Geometry check sheet. Reference: the model listing, model coordinates, mm. A direction names the side the tool comes from. Give positions to 0.01 mm unless a question says otherwise; leave off trailing zeros. Loops run counter-clockwise (first coordinate to the right, second up) from the corner with the lowest first, then second, coordinate; pieces in that order, holes last. Notation, with made-up numbers: (-28, 65) - (26, 65) arc R26 cw to (26, 94) - close; hole circle Ø7 at (-18, -14.5). An arc over 180 degrees is marked (long way). Write item = value, one per line. Start each with the question number.
from build123d import *

# Parameters (mm, degrees)
SKETCH_1_W            = 90
SKETCH_1_H            = 25
EXTRUDE_1_DEPTH       = 12
SKETCH_2_W            = 40
SKETCH_2_H            = 25
EXTRUDE_2_DEPTH       = 35
HOLE_WIZARD_M20_1_D   = 17.5
HOLE_WIZARD_9_0_9_1_D = 9
CHAMFER_1_SIZE        = 5
CHAMFER_2_SIZE        = 3


with BuildPart() as part:
    # 草图1 → 凸台-拉伸1 (new body)
    with BuildSketch(Plane(origin=(0, 0, 0), x_dir=(0, 0, -1), z_dir=(1, 0, 0))):
        Rectangle(SKETCH_1_W, SKETCH_1_H)
    extrude(amount=EXTRUDE_1_DEPTH)

    # 草图2 → 凸台-拉伸2 (add)
    with BuildSketch(Plane(origin=(12, 0, 0), x_dir=(0, 0, -1), z_dir=(1, 0, 0))):
        Rectangle(SKETCH_2_W, SKETCH_2_H)
    extrude(amount=EXTRUDE_2_DEPTH)

    # M20 螺纹孔1 (through all)
    with Locations(Plane(origin=(0, -12.5, 0), x_dir=(-1, 0, 0), z_dir=(0, -1, 0))):
        with Locations((-30, 0)):
            Hole(HOLE_WIZARD_M20_1_D / 2)

    # Ø9.0 (9) 直径孔1 (through all)
    with Locations(Plane(origin=(12, 0, 0), x_dir=(0, 0, -1), z_dir=(1, 0, 0))):
        with Locations((-30, 0), (30, 0)):
            Hole(HOLE_WIZARD_9_0_9_1_D / 2)

    # 倒角1
    chamfer_1_edges = [part.edges().sort_by_distance(p)[0] for p in [
        (47, 0, -20),
        (47, 0, 20),
    ]]
    chamfer(chamfer_1_edges, length=CHAMFER_1_SIZE)

    # 倒角2
    chamfer_2_edges = [part.edges().sort_by_distance(p)[0] for p in [
        (6, -12.5, -45),
        (6, -12.5, 45),
        (6, 12.5, 45),
        (6, 12.5, -45),
    ]]
    chamfer(chamfer_2_edges, length=CHAMFER_2_SIZE)


solid = part.part
1) Material ranges on line 1 along Z through (x, y) = (30, -0.5); line 2 along Y through (x, z) = (8.75, -30); line 3 along Z through (x, y) = (6.5, -4), recorded low to high.
2) Cross-section at A-A on y = 0. Enter the section's corners in (x, z), and give its area (3 significant figures).
3) Cross-section at C-C on x = 28.5. Enter the section's corners in (y, z).
4) Release check for a two-part mould opening along Y. For faces 1 (the face through (5.916, 1.352, 34.292)), 2 (the face through (27, 0, -20)), 3 (the face through (18, 12.5, 1)) record: pulls with the +Y half, pulls with the -Y half, needs draft (parallel to the pull), parting line crosses it, or undercut.
5) Cross-section at B-B on z = 30. Enter the section's corners in (x, y), and give its area (3 significant figures).
6) Cross-section at D-D on x = 3. Enter the section's corners in (y, z), and give its area (3 significant figures).
7) Tool access check on faces 4 (the face through (27, 0, 20)), 5 (the face through (12, 0, -35)), 6 (the face through (6, 0, 45)). Record the directions out of +Z, -Z, +X, -X, +Y, -Y that give a thin tool (end or side, any length) a straight path to the whole face; none if there is none.
8) Gauge pin test, flat ends, axial feed: P1, Ø1, axis at x = 24, y = 2, coming from the +Z side; P2, Ø4, axis at x = 38, y = -2, coming from the -Z side; P3, Ø1.5, axis at y = 1, z = -22.5, coming from the +X side. Record the tip position at first contact, or that the pin passes through.
Checked values:
q1.line_1 = -20 to -8.75, 8.75 to 20
q1.line_2 = -12.5 to -4.5, 4.5 to 12.5
q1.line_3 = -45 to -32.06, -27.94 to 27.94, 32.06 to 45
q2.outline = (0, -45) - (12, -45) - (12, -34.5) - (0, -34.5) - close; (0, -25.5) - (12, -25.5) - (12, -20) - (42, -20) - (47, -15) - (47, 15) - (42, 20) - (12, 20) - (12, 25.5) - (0, 25.5) - close; (0, 34.5) - (12, 34.5) - (12, 45) - (0, 45) - close; hole circle Ø17.5 at (30, 0)
q2.area = 2,000 mm²
q3.outline = (-12.5, -20) - (12.5, -20) - (12.5, -8.62) - (-12.5, -8.62) - close; (-12.5, 8.62) - (12.5, 8.62) - (12.5, 20) - (-12.5, 20) - close
q4.face_1 = undercut
q4.face_2 = needs draft
q4.face_3 = pulls with the +Y half
q5.outline = (0, -12.5) - (12, -12.5) - (12, -4.5) - (0, -4.5) - close; (0, 4.5) - (12, 4.5) - (12, 12.5) - (0, 12.5) - close
q5.area = 192 mm²
q6.outline = (-12.5, -42) - (-9.5, -45) - (9.5, -45) - (12.5, -42) - (12.5, 42) - (9.5, 45) - (-9.5, 45) - (-12.5, 42) - close; hole circle Ø9 at (0, -30); hole circle Ø9 at (0, 30)
q6.area = 2,100 mm²
q7.face_4 = +Z, +X, +Y, -Y
q7.face_5 = -Z, +X, +Y, -Y
q7.face_6 = +Z, +X, -X, +Y, -Y
q8.P1 = 20
q8.P2 = -20
q8.P3 = 12
